The model under review builds one solid part; all positions refer to its coordinate system, in mm. A direction names the side the tool comes from. Coordinates: 2 decimals unless noted, no trailing zeros. Write each loop counter-clockwise with the first axis right and the second up, starting at its lowest first coordinate (ties: lowest second). Pieces come first, ordered by that corner, then holes.
```python
from build123d import *

# Parameters (mm, degrees)
BASE_BLOCK_100X100X30_DEPTH        = 15
LOCATING_PADS_10MM_DEPTH           = 10
LOCATING_PAD_FILLET_R15_1_R        = 15
LOCATING_PAD_FILLET_R15_2_R        = 15
LOCATING_PAD_FILLET_R15_3_R        = 15
LOCATING_PAD_FILLET_R15_4_R        = 15
RAISED_PAD_10MM_DEPTH              = 10
RAISED_PAD_FILLET_R10_1_R          = 10
RAISED_PAD_FILLET_R10_2_R          = 10
RAISED_PAD_FILLET_R10_3_R          = 10
RAISED_PAD_FILLET_R10_4_R          = 10
RAISED_PAD_POCKET_SKETCH_R         = 5
RAISED_PAD_POCKET_10X10X10_DEPTH   = 10
LOCATING_PAD_POCKET_SKETCH_R       = 7.5
LOCATING_PAD_POCKET_15X15X10_DEPTH = 10


with BuildPart() as part:
    # Base Block Sketch → Base Block 100x100x30 (new, symmetric)
    with BuildSketch(Plane.XY):
        Polygon((50, 45), (-50, 45), (-50, -55), (50, -55), (50, 0), align=None)
    extrude(amount=BASE_BLOCK_100X100X30_DEPTH, both=True)

    # Locating Pads Sketch → Locating Pads 10mm (add)
    with BuildSketch(Plane(origin=(0, 0, -15), x_dir=(-1, 0, 0), z_dir=(0, 0, -1))):
        with BuildLine():
            Line((15, 40), (45, 40))
            Line((45, 40), (45, 10))
            ThreePointArc((45, 10), (30, -5), (45, -20))
            Line((45, -20), (45, -50))
            Line((45, -50), (15, -50))
            ThreePointArc((15, -50), (0, -35), (-15, -50))
            Line((-15, -50), (-45, -50))
            Line((-45, -50), (-45, -20))
            ThreePointArc((-45, -20), (-30, -5), (-45, 10))
            Line((-45, 10), (-45, 40))
            Line((-45, 40), (-15, 40))
            ThreePointArc((-15, 40), (0, 25), (15, 40))
        make_face()
    extrude(amount=LOCATING_PADS_10MM_DEPTH)

    # Locating Pad Fillet R15 1
    locating_pad_fillet_r15_1_edges = [part.edges().sort_by_distance(p)[0] for p in [
        (-45, -50, -20),
    ]]
    fillet(locating_pad_fillet_r15_1_edges, radius=LOCATING_PAD_FILLET_R15_1_R)

    # Locating Pad Fillet R15 2
    locating_pad_fillet_r15_2_edges = [part.edges().sort_by_distance(p)[0] for p in [
        (45, -50, -20),
    ]]
    fillet(locating_pad_fillet_r15_2_edges, radius=LOCATING_PAD_FILLET_R15_2_R)

    # Locating Pad Fillet R15 3
    locating_pad_fillet_r15_3_edges = [part.edges().sort_by_distance(p)[0] for p in [
        (45, 40, -20),
    ]]
    fillet(locating_pad_fillet_r15_3_edges, radius=LOCATING_PAD_FILLET_R15_3_R)

    # Locating Pad Fillet R15 4
    locating_pad_fillet_r15_4_edges = [part.edges().sort_by_distance(p)[0] for p in [
        (-45, 40, -20),
    ]]
    fillet(locating_pad_fillet_r15_4_edges, radius=LOCATING_PAD_FILLET_R15_4_R)

    # Raised Pad Sketch → Raised Pad 10mm (add)
    with BuildSketch(Plane(origin=(0, 0, -25), x_dir=(-1, 0, 0), z_dir=(0, 0, -1))):
        Polygon((0, -25), (20, -25), (20, 15), (-20, 15), (-20, -25), align=None)
    extrude(amount=RAISED_PAD_10MM_DEPTH)

    # Raised Pad Fillet R10 1
    raised_pad_fillet_r10_1_edges = [part.edges().sort_by_distance(p)[0] for p in [
        (20, -25, -30),
    ]]
    fillet(raised_pad_fillet_r10_1_edges, radius=RAISED_PAD_FILLET_R10_1_R)

    # Raised Pad Fillet R10 2
    raised_pad_fillet_r10_2_edges = [part.edges().sort_by_distance(p)[0] for p in [
        (20, 15, -30),
    ]]
    fillet(raised_pad_fillet_r10_2_edges, radius=RAISED_PAD_FILLET_R10_2_R)

    # Raised Pad Fillet R10 3
    raised_pad_fillet_r10_3_edges = [part.edges().sort_by_distance(p)[0] for p in [
        (-20, 15, -30),
    ]]
    fillet(raised_pad_fillet_r10_3_edges, radius=RAISED_PAD_FILLET_R10_3_R)

    # Raised Pad Fillet R10 4
    raised_pad_fillet_r10_4_edges = [part.edges().sort_by_distance(p)[0] for p in [
        (-20, -25, -30),
    ]]
    fillet(raised_pad_fillet_r10_4_edges, radius=RAISED_PAD_FILLET_R10_4_R)

    # Raised Pad Pocket Sketch → Raised Pad Pocket 10x10x10 (cut)
    with BuildSketch(Plane(origin=(0, 0, -35), x_dir=(-1, 0, 0), z_dir=(0, 0, -1))):
        with Locations((10, 5)):
            Circle(RAISED_PAD_POCKET_SKETCH_R)
        with Locations((10, -15)):
            Circle(RAISED_PAD_POCKET_SKETCH_R)
        with Locations((-10, -15)):
            Circle(RAISED_PAD_POCKET_SKETCH_R)
        with Locations((-10, 5)):
            Circle(RAISED_PAD_POCKET_SKETCH_R)
    extrude(amount=-RAISED_PAD_POCKET_10X10X10_DEPTH, mode=Mode.SUBTRACT)

    # Locating Pad Pocket Sketch → Locating Pad Pocket 15x15x10 (cut)
    with BuildSketch(Plane(origin=(0, 0, -25), x_dir=(-1, 0, 0), z_dir=(0, 0, -1))):
        with Locations((30, 25)):
            Circle(LOCATING_PAD_POCKET_SKETCH_R)
        with Locations((30, -35)):
            Circle(LOCATING_PAD_POCKET_SKETCH_R)
        with Locations((-30, -35)):
            Circle(LOCATING_PAD_POCKET_SKETCH_R)
        with Locations((-30, 25)):
            Circle(LOCATING_PAD_POCKET_SKETCH_R)
    extrude(amount=-LOCATING_PAD_POCKET_15X15X10_DEPTH, mode=Mode.SUBTRACT)


solid = part.part
```
Item 1: Mouldability with a two-part tool opening along X and no side actions: class faces 1 (the face through (-28.37, -42.32, -20.07)), 2 (the face through (40.72, 35.49, -20.07)), 3 (the face through (31.63, -42.32, -20.07)), 4 (the face through (0, 15, -30)) as pulls with the +X half, pulls with the -X half, needs draft (parallel to the pull), parting line crosses it, or undercut.
Solved:
face 1: undercut
face 2: pulls with the +X half
face 3: undercut
face 4: needs draft
Item 2: Take a section at A-A, the plane z = -28. Write out the cut boundary in (x, y), plus the area to 3 significant figures.
Solved:
outline: (-20, -15) arc R10 ccw to (-10, -25) - (10, -25) arc R10 ccw to (20, -15) - (20, 5) arc R10 ccw to (10, 15) - (-10, 15) arc R10 ccw to (-20, 5) - close; hole circle Ø10 at (-10, -15); hole circle Ø10 at (-10, 5); hole circle Ø10 at (10, -15); hole circle Ø10 at (10, 5)
area: 1,200 mm2
Item 3: To check wall thickness, follow line 1 along Z through (x, y) = (-42.5, 30.5); line 2 along Z through (x, y) = (-32, -6); line 3 along X through (y, z) = (36, -23). State the ranges of each line that lie inside material, in increasing order.
Solved:
line 1: z = -25 to 15
line 2: z = -15 to 15
line 3: x = -40.2 to -14.46, 14.46 to 40.2
Item 4: For pin 1 (11 mm diameter, centred on x = 26, z = -22.5, fed in from -Y); pin 2 (5 mm diameter, centred on x = -21.5, z = -20, fed in from +Y); pin 3 (4.5 mm diameter, centred on x = -33, y = 28.5, fed in from -Z); pin 4 (6 mm diameter, centred on x = 0.5, z = -17.5, fed in from +Y), all flat-tipped, find the tip position at first contact; note any pin that passes through.
Solved:
pin 1: stops at y = -50
pin 2: stops at y = 40
pin 3: stops at z = -15
pin 4: stops at y = 45
Item 5: Take a section at C-C, the plane y = -5.5. Write out the cut boundary in (x, z).
Solved:
outline: (-50, -15) - (-30.01, -15) - (-30.01, -25) - (-20, -25) - (-20, -35) - (20, -35) - (20, -25) - (30.01, -25) - (30.01, -15) - (50, -15) - (50, 15) - (-50, 15) - close
Item 6: Machinability: for faces 5 (the face through (0, -25, -30)), 6 (the face through (-30, -5, -20)), 7 (the face through (-12.307, -19.436, -30.07)), which of the approach directions +Z, -Z, +X, -X, +Y, -Y give a long, thin tool a straight path to every point of the face, cutting with its end or side? Answer none if there is none.
Solved:
face 5: -Z, +X, -X, -Y
face 6: -Z, -X
face 7: -Z
Item 7: Take a section at D-D, the plane y = -17. Write out the cut boundary in (x, z).
Solved:
outline: (-50, -15) - (-36, -15) - (-36, -25) - (-19.8, -25) - (-19.8, -35) - (-14.58, -35) - (-14.58, -25) - (-5.42, -25) - (-5.42, -35) - (5.42, -35) - (5.42, -25) - (14.58, -25) - (14.58, -35) - (19.8, -35) - (19.8, -25) - (36, -25) - (36, -15) - (50, -15) - (50, 15) - (-50, 15) - close
Item 8: Take a section at B-B, the plane x = 0. Write out the cut boundary in (y, z), plus the area to 3 significant figures.
Solved:
outline: (-55, -15) - (-35, -15) - (-35, -25) - (-25, -25) - (-25, -35) - (15, -35) - (15, -25) - (25, -25) - (25, -15) - (45, -15) - (45, 15) - (-55, 15) - close
area: 4,000 mm2
